Check sheet for the modelled part. Datum: model origin and axes. Units: mm. Face numbers are marked on the shaded views. A direction names the side the tool comes from. Round coordinates to 2 decimals unless told otherwise and drop trailing zeros. Write each loop counter-clockwise with the first axis right and the second up, starting at its lowest first coordinate (ties: lowest second). Pieces come first, ordered by that corner, then holes. Notation, with made-up numbers: (45.5, 20) -> (97.5, 20) arc R22 ccw to (97.5, 40) -> close; hole circle Ø9 at (27.5, 18.5). An arc over 180 degrees is marked (long way). Answer as a JSON object with one key per item and string values. Group by question number.
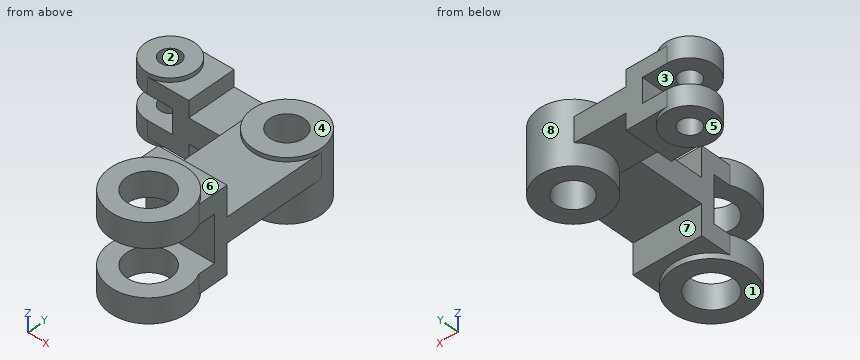
```python
from build123d import *

# Parameters (mm, degrees)
FRONT_PIVOT_EYE_SKETCH_R        = 28
FRONT_PIVOT_EYE_SKETCH_R_2      = 16
FRONT_PIVOT_EYE_56X_32_DEPTH    = 18
REAR_PIVOT_EYE_SKETCH_R         = 28
REAR_PIVOT_EYE_SKETCH_R_2       = 16
REAR_PIVOT_EYE_56X_32_DEPTH     = 18
LOWER_CLEVIS_BLOCK_48X48_DEPTH  = 18
CLEVIS_BLOCK_RELIEF_SKETCH_W    = 3
CLEVIS_BLOCK_RELIEF_SKETCH_H    = 18
CLEVIS_BLOCK_RELIEF_CUT_DEPTH   = 80.780950107
LOWER_CLEVIS_SLOT_SKETCH_W      = 34
LOWER_CLEVIS_SLOT_SKETCH_H      = 8
LOWER_CLEVIS_SLOT_34X8_DEPTH    = 95.519839187
LOWER_WEB_PLATE_SKETCH_W        = 2.751404539
LOWER_WEB_PLATE_SKETCH_H        = 14
LOWER_WEB_PLATE_SKETCH_W_2      = 2.75570227
LOWER_WEB_PLATE_5MM_DEPTH       = 5
MAIN_ARM_SKETCH_W               = 50.004297731
MAIN_ARM_SKETCH_H               = 18
MAIN_ARM_9X18_DEPTH             = 75
UPPER_PIVOT_HUB_SKETCH_R        = 25
UPPER_PIVOT_HUB_SKETCH_R_2      = 12.5
UPPER_PIVOT_HUB_50X_25_DEPTH    = 46
HUB_BORE_SKETCH_R               = 12.5
HUB_BORE_THROUGH_CUT_25_DEPTH   = 145.723875017
UPPER_ARM_SKETCH_R              = 18
UPPER_ARM_SKETCH_R_2            = 7.5
UPPER_ARM_36X15_DEPTH           = 15
UPPER_ARM_EXTENSION_SKETCH_R    = 18
UPPER_ARM_EXTENSION_SKETCH_R_2  = 7.5
UPPER_ARM_EXTENSION_36X15_DEPTH = 15
UPPER_CLEVIS_HEAD_DEPTH         = 36
UPPER_CLEVIS_SLOT_SKETCH_R      = 12.5
UPPER_CLEVIS_SLOT_SKETCH_R_2    = 7.5
UPPER_CLEVIS_SLOT_25_DEPTH      = 177.188981887


with BuildPart() as part:
    # Front Pivot Eye Sketch → Front Pivot Eye Ø56xØ32 (new body)
    with BuildSketch(Plane.XY):
        Circle(FRONT_PIVOT_EYE_SKETCH_R)
        Circle(FRONT_PIVOT_EYE_SKETCH_R_2, mode=Mode.SUBTRACT)
    extrude(amount=-FRONT_PIVOT_EYE_56X_32_DEPTH)



with BuildPart() as body_2:
    # Rear Pivot Eye Sketch → Rear Pivot Eye Ø56xØ32 (new body)
    with BuildSketch(Plane.XY.offset(-52)):
        Circle(REAR_PIVOT_EYE_SKETCH_R)
        Circle(REAR_PIVOT_EYE_SKETCH_R_2, mode=Mode.SUBTRACT)
    extrude(amount=-REAR_PIVOT_EYE_56X_32_DEPTH)


with BuildPart() as part_1:
    add(part.part)

    add(body_2.part)  # Lower Clevis Block 48x48 merges body 2
    # Lower Clevis Block Sketch → Lower Clevis Block 48x48 (add)
    with BuildSketch(Plane(origin=(0, 35, 0), x_dir=(1, 0, 0), z_dir=(0, 1, 0))):
        Polygon((-28, 52), (-28, 66), (28, 66), (28, 18), (28, 4), (-28, 4), align=None)
    extrude(amount=-LOWER_CLEVIS_BLOCK_48X48_DEPTH)

    # Clevis Block Relief Sketch → Clevis Block Relief Cut (cut, through all)
    with BuildSketch(Plane.XY.offset(-4)):
        with Locations((-26.5, 26)):
            Rectangle(CLEVIS_BLOCK_RELIEF_SKETCH_W, CLEVIS_BLOCK_RELIEF_SKETCH_H)
        Polygon((28, 17), (25.124297731, 17), (25.004297731, 17), (25.004297731, 35), (28, 35), align=None)
    extrude(amount=-CLEVIS_BLOCK_RELIEF_CUT_DEPTH, mode=Mode.SUBTRACT)

    # Lower Clevis Slot Sketch → Lower Clevis Slot 34x8 (cut, through all)
    with BuildSketch(Plane.ZY.offset(25)):
        with Locations((-35, 21)):
            Rectangle(LOWER_CLEVIS_SLOT_SKETCH_W, LOWER_CLEVIS_SLOT_SKETCH_H)
    extrude(amount=-LOWER_CLEVIS_SLOT_34X8_DEPTH, mode=Mode.SUBTRACT)

    # Lower Web Plate Sketch → Lower Web Plate 5mm (add)
    with BuildSketch(Plane.XZ.offset(-17)):
        with Locations((-23.624297731, -59)):
            Rectangle(LOWER_WEB_PLATE_SKETCH_W, LOWER_WEB_PLATE_SKETCH_H)
        with Locations((-23.624297731, -11)):
            Rectangle(LOWER_WEB_PLATE_SKETCH_W, LOWER_WEB_PLATE_SKETCH_H)
        with Locations((23.626446596, -11)):
            Rectangle(LOWER_WEB_PLATE_SKETCH_W_2, LOWER_WEB_PLATE_SKETCH_H)
        with Locations((23.626446596, -59)):
            Rectangle(LOWER_WEB_PLATE_SKETCH_W_2, LOWER_WEB_PLATE_SKETCH_H)
    extrude(amount=LOWER_WEB_PLATE_5MM_DEPTH)

    # Main Arm Sketch → Main Arm 9x18 (add)
    with BuildSketch(Plane(origin=(0, 35, 0), x_dir=(1, 0, 0), z_dir=(0, 1, 0))):
        with Locations((0.002148866, 35)):
            Rectangle(MAIN_ARM_SKETCH_W, MAIN_ARM_SKETCH_H)
    extrude(amount=MAIN_ARM_9X18_DEPTH)

    # Upper Pivot Hub Sketch → Upper Pivot Hub Ø50xØ25 (add)
    with BuildSketch(Plane.XY.offset(-23)):
        with Locations((0.002148865, 110)):
            Circle(UPPER_PIVOT_HUB_SKETCH_R)
        with Locations((0.002148865, 110)):
            Circle(UPPER_PIVOT_HUB_SKETCH_R_2, mode=Mode.SUBTRACT)
    extrude(amount=-UPPER_PIVOT_HUB_50X_25_DEPTH)

    # Hub Bore Sketch → Hub Bore Through Cut Ø25 (cut, through all)
    with BuildSketch(Plane.XY.offset(-26)):
        with Locations((0.002148865, 110)):
            Circle(HUB_BORE_SKETCH_R)
    extrude(amount=-HUB_BORE_THROUGH_CUT_25_DEPTH, mode=Mode.SUBTRACT)



with BuildPart() as body_2_2:
    # Upper Arm Sketch → Upper Arm 36x15 (new body)
    with BuildSketch(Plane.XY.offset(-20)):
        with Locations((-84.997851135, 110)):
            Circle(UPPER_ARM_SKETCH_R)
        with Locations((-84.997851135, 110)):
            Circle(UPPER_ARM_SKETCH_R_2, mode=Mode.SUBTRACT)
    extrude(amount=-UPPER_ARM_36X15_DEPTH)


with BuildPart() as body_3:
    # Upper Arm Extension Sketch → Upper Arm Extension 36x15 (new body)
    with BuildSketch(Plane.XY.offset(-53)):
        with Locations((-84.997851135, 110)):
            Circle(UPPER_ARM_EXTENSION_SKETCH_R)
        with Locations((-84.997851135, 110)):
            Circle(UPPER_ARM_EXTENSION_SKETCH_R_2, mode=Mode.SUBTRACT)
    extrude(amount=-UPPER_ARM_EXTENSION_36X15_DEPTH)


with BuildPart() as part_2:
    add(part_1.part)

    add(body_2_2.part)  # Upper Clevis Head merges body 2 2

    add(body_3.part)  # Upper Clevis Head merges body 3
    # Upper Clevis Head Sketch → Upper Clevis Head (add)
    with BuildSketch(Plane(origin=(0, 128, 0), x_dir=(1, 0, 0), z_dir=(0, 1, 0))):
        Polygon((-84.997851135, 53), (-84.997851135, 65), (-54.997851135, 65), (-54.997851135, 53), (-4.745708578, 53), (-4.745708578, 35), (-54.997851135, 35), (-54.997851135, 23), (-84.997851135, 23), (-84.997851135, 35), (-66.997851135, 35), (-66.997851135, 53), align=None)
    extrude(amount=-UPPER_CLEVIS_HEAD_DEPTH)

    # Upper Clevis Slot Sketch → Upper Clevis Slot 25 (cut, through all)
    with BuildSketch(Plane.XY.offset(-23)):
        with Locations((0.002148865, 110)):
            Circle(UPPER_CLEVIS_SLOT_SKETCH_R)
        with Locations((-84.997851135, 110)):
            Circle(UPPER_CLEVIS_SLOT_SKETCH_R_2)
    extrude(amount=-UPPER_CLEVIS_SLOT_25_DEPTH, mode=Mode.SUBTRACT)


solid = part_2.part
```
(1) Section check B-B on z = -60.5. Record the cut outline in (x, y).
(2) Go/stop test with flat-tipped pins: pin 1 Ø15 at (x, y) = (-70.5, 112) entering from -Z; pin 2 Ø21 at (x, z) = (-56.5, -40) entering from -Y; pin 3 Ø17.5 at (x, z) = (4, -13) entering from +Y. Record where each tip stops, or that it passes through.
(3) Release check for a two-part mould opening along Z. For the marked faces 1, 2, 3 and 4 record: pulls with the +Z half, pulls with the -Z half, needs draft (parallel to the pull), parting line crosses it, or undercut.
(4) Scan lines: line 1 along Y through (x, z) = (0, -61.5); line 2 along Y through (x, z) = (0, -13); line 3 along Z through (x, y) = (-20, -2.5). Record each from-to range of solid material in increasing order.
(5) Section check C-C on y = 0. Record the cut outline in (x, z), then the cut area to 3 significant figures.
(6) Access from +Z, -Z, +X, -X, +Y, -Y to the whole of each face (thin tool, end or side, straight path). Record for the marked faces 5, 6, 7 and 8.
(7) Section check A-A on x = 0. State how many separate pieces and enclosed holes the cut face has, then the cut area to 3 significant figures.
(8) Section check D-D on z = -50. Record the cut outline in (x, y), then the cut area to 3 significant figures.
Data:
{
 "1": {"outline": "(-85, 92) -> (-55, 92) -> (-55, 128) -> (-85, 128) arc R18 ccw to start; (-25, 12.61) arc R28 ccw (long way) to (25, 12.6) -> (25, 35) -> (-25, 35) -> close; circle Ø50 at (0, 110); hole circle Ø15 at (-85, 110); hole circle Ø32 at (0, 0); hole circle Ø25 at (0, 110)"},
 "2": {"pin 1": "stops at z = -68", "pin 2": "stops at y = 92", "pin 3": "stops at y = 35"},
 "3": {"face 1": "pulls with the -Z half", "face 2": "needs draft", "face 3": "undercut", "face 4": "pulls with the +Z half"},
 "4": {"line 1": "y = -28 to -16, 16 to 35, 85 to 97.5, 122.5 to 135", "line 2": "y = -28 to -16, 16 to 35", "line 3": "z = -70 to -52, -18 to 0"},
 "5": {"outline": "(-28, -70) -> (-16, -70) -> (-16, -52) -> (-28, -52) -> close; (-28, -18) -> (-16, -18) -> (-16, 0) -> (-28, 0) -> close; (16, -70) -> (28, -70) -> (28, -52) -> (16, -52) -> close; (16, -18) -> (28, -18) -> (28, 0) -> (16, 0) -> close", "area": "864 mm²"},
 "6": {"face 5": "-Z, -X, +Y, -Y", "face 6": "+Z, +Y", "face 7": "-Z, +X, -X", "face 8": "none"},
 "7": {"separate pieces": "4", "enclosed holes": "0", "area": "3,450 mm²"},
 "8": {"outline": "(-67, 92) -> (-17.35, 92) arc R25 ccw (long way) to (-17.35, 128) -> (-67, 128) -> close; (-25, 25) -> (25, 25) -> (25, 35) -> (-25, 35) -> close; hole circle Ø25 at (0, 110)", "area": "3,570 mm²"}
}
